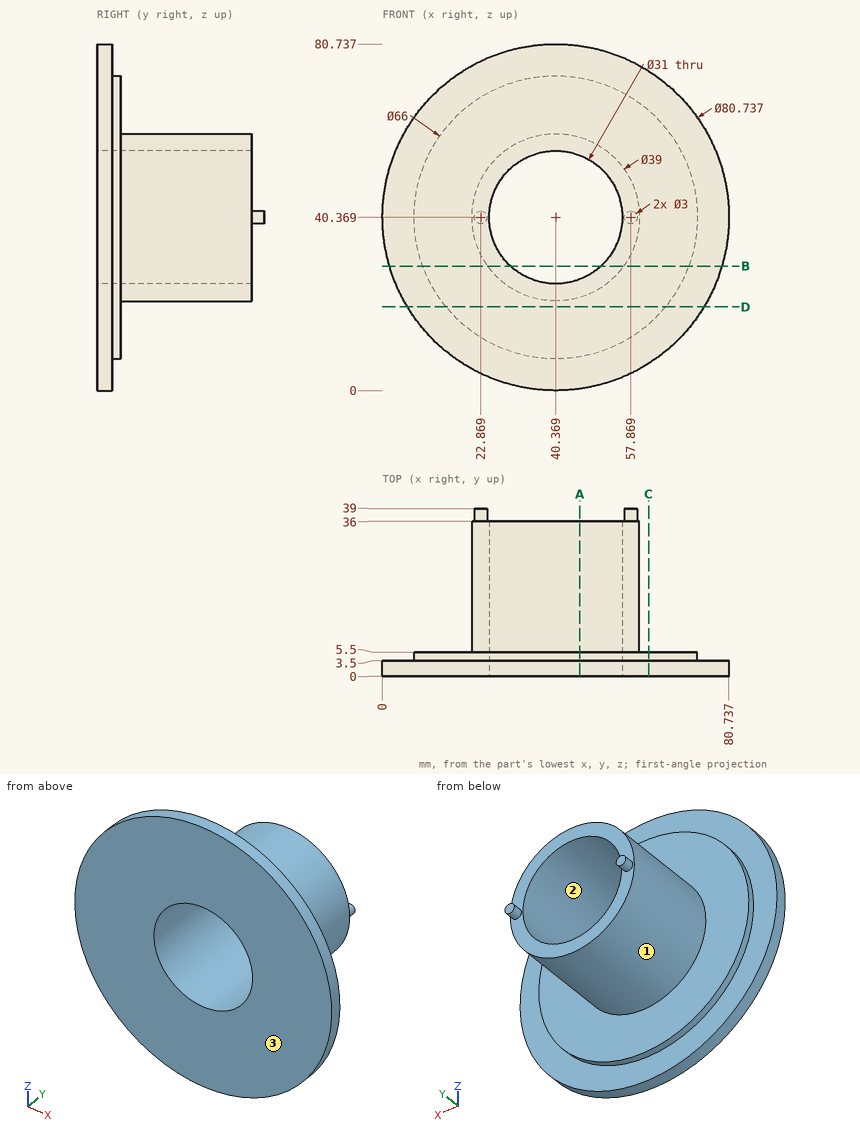
The drawing under review shows one solid part. Ordinate dimensions are in mm from its lowest x, y, z. Coordinates: 2 decimals unless noted, no trailing zeros. Write each loop counter-clockwise with the first axis right and the second up, starting at its lowest first coordinate (ties: lowest second). Pieces come first, ordered by that corner, then holes. Notation, with made-up numbers: (-9.5, -39) - (44.5, -39) arc R17 cw to (44.5, -24) - close; hole circle Ø6 at (65, 45.5). An arc over 180 degrees is marked (long way). Put each result on its own line as item: value.
1. Mouldability with a two-part tool opening along X and no side actions: class the marked faces 1, 2 and 3 as released by +X, released by -X, zero draft, split by the parting line, or undercut.
Values found:
face 1: split by the parting line
face 2: undercut
face 3: zero draft
2. For pin 1 (1.5 mm diameter, centred on x = 10.5, z = 25.5, fed in from +Y); pin 2 (25 mm diameter, centred on x = 40.37, z = 40.37, fed in from +Y); pin 3 (5 mm diameter, centred on x = 32.5, z = 22.5, fed in from +Y); pin 4 (24 mm diameter, centred on x = 51, z = 45.5, fed in from +Y), all flat-tipped, find the tip position at first contact; note any pin that passes through.
Values found:
pin 1: y = 5.5
pin 2: through
pin 3: y = 36
pin 4: y = 39
3. Add section C-C, the plane x = 62. Give the boundary of the cut face in (y, z) (1 decimal), then the cut area to 3 significant figures.
Values found:
outline: (0, 6.3) - (3.5, 6.3) - (3.5, 15.4) - (5.5, 15.4) - (5.5, 65.3) - (3.5, 65.3) - (3.5, 74.5) - (0, 74.5) - close
area: 338 mm²
4. Wall thickness on probe 1 along Y at (x, z) = (54, 48); probe 2 along Y at (x, z) = (10.5, 49); probe 3 along Z at (x, y) = (32, 13.5) (1 decimal): over which ranges is each line inside the solid? List them lowest first.
Values found:
probe 1: 0 to 36
probe 2: 0 to 5.5
probe 3: 22.8 to 27.3, 53.4 to 58
5. Add section D-D, the plane z = 19.5. Give the boundary of the cut face in (x, y) (1 decimal), then the cut area to 3 significant figures.
Values found:
outline: (5.8, 0) - (74.9, 0) - (74.9, 3.5) - (65.9, 3.5) - (65.9, 5.5) - (14.8, 5.5) - (14.8, 3.5) - (5.8, 3.5) - close
area: 344 mm²
6. Add section A-A, the plane x = 46. Give the boundary of the cut face in (y, z) (1 decimal).
Values found:
outline: (0, 0.4) - (3.5, 0.4) - (3.5, 7.9) - (5.5, 7.9) - (5.5, 21.7) - (36, 21.7) - (36, 25.9) - (0, 25.9) - close; (0, 54.8) - (36, 54.8) - (36, 59) - (5.5, 59) - (5.5, 72.9) - (3.5, 72.9) - (3.5, 80.3) - (0, 80.3) - close
7. Add section B-B, the plane z = 29. Give the boundary of the cut face in (x, y) (1 decimal), then the cut area to 3 significant figures.
Values found:
outline: (1.6, 0) - (29.8, 0) - (29.8, 36) - (24.5, 36) - (24.5, 5.5) - (9.4, 5.5) - (9.4, 3.5) - (1.6, 3.5) - close; (50.9, 0) - (79.1, 0) - (79.1, 3.5) - (71.3, 3.5) - (71.3, 5.5) - (56.2, 5.5) - (56.2, 36) - (50.9, 36) - close
area: 603 mm²
